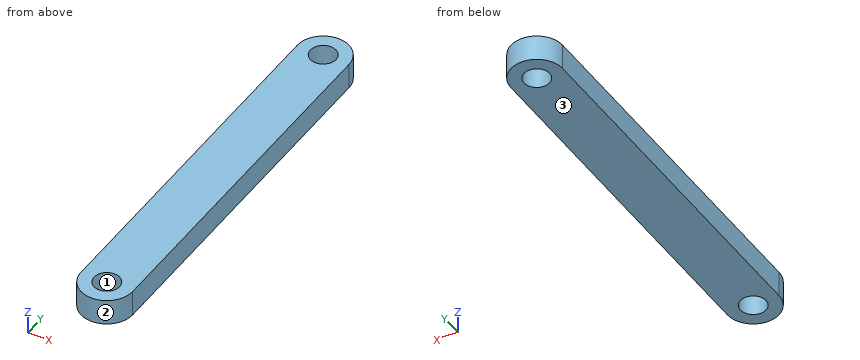
```python
from build123d import *

# Parameters (mm, degrees)
SKETCH1_R           = 1.59
BOSS_EXTRUDE1_DEPTH = 3.18
SCALE_RATIO_1_SCALE = 1.3


with BuildPart() as part:
    # Sketch1 → Boss-Extrude1 (new body)
    with BuildSketch(Plane.XY):
        with BuildLine():
            Line((-3.2, 0), (-3.2, 45))
            ThreePointArc((-3.2, 45), (0, 48.2), (3.2, 45))
            Line((3.2, 45), (3.2, 0))
            ThreePointArc((3.2, 0), (0, -3.2), (-3.2, 0))
        make_face()
        with Locations(Location((0, 0, 0), (0, 0, 180))):
            Circle(SKETCH1_R, mode=Mode.SUBTRACT)
        with Locations(Location((0, 45, 0), (0, 0, 180))):
            Circle(SKETCH1_R, mode=Mode.SUBTRACT)
    extrude(amount=BOSS_EXTRUDE1_DEPTH)


with BuildPart() as part_1:
    # Scale ratio 1: scaled about (0, 0, 0)
    add(part.part.scale(SCALE_RATIO_1_SCALE))


solid = part_1.part
```
CAD build for the part. Positions are in the model's coordinates, mm. Face numbers are marked on the shaded views. Coordinates: 2 decimals unless noted, no trailing zeros. Loops run counter-clockwise (first coordinate to the right, second up) from the corner with the lowest first, then second, coordinate; pieces in that order, holes last. Notation, with made-up numbers: (-21.5, 73) - (31.5, 73) arc R23 cw to (31.5, 112) - close; hole circle Ø1 at (-29, 9). An arc over 180 degrees is marked (long way). Use CSV: the item, a comma, the result in double quotes. Start each with the question number.
Q1. Two-plate mould, pull along Y, no slides. Class the marked faces 1, 2 and 3: +Y half, -Y half, draft (parallel to the pull), parting line (faces both ways), or undercut.
Q2. Cut at A-A, the plane x = 0. List the corners of the cut face in (y, z), then the cut area to 3 significant figures.
Q3. Cut at B-B, the plane z = 2.85. List the corners of the cut face in (x, y), then the cut area to 3 significant figures.
Q4. Probe probe 1 along Y at (x, z) = (0, 3.1); probe 2 along X at (y, z) = (58.5, 2.55); probe 3 along Y at (x, z) = (-1, 0.85). List the from-to ranges inside material, lowest first. Write a range as from..to.
Here are the results:
1,face 1,"undercut"
1,face 2,"-Y half"
1,face 3,"draft"
2,outline,"(-4.16, 0) - (-2.07, 0) - (-2.07, 4.13) - (-4.16, 4.13) - close; (2.07, 0) - (56.43, 0) - (56.43, 4.13) - (2.07, 4.13) - close; (60.57, 0) - (62.66, 0) - (62.66, 4.13) - (60.57, 4.13) - close"
2,area,"242 mm2"
3,outline,"(-4.16, 0) arc R4.16 ccw to (4.16, 0) - (4.16, 58.5) arc R4.16 ccw to (-4.16, 58.5) - close; hole circle Ø4.13 at (0, 0); hole circle Ø4.13 at (0, 58.5)"
3,area,"514 mm2"
4,probe 1,"-4.16..-2.07, 2.07..56.43, 60.57..62.66"
4,probe 2,"-4.16..-2.07, 2.07..4.16"
4,probe 3,"-4.04..-1.81, 1.81..56.69, 60.31..62.54"
